Work out the finished part from the listing and answer in its coordinate system (mm). Face numbers are marked on the shaded views. A direction names the side the tool comes from. Coordinates: 2 decimals unless noted, no trailing zeros. Order: outer loops, then holes, each group sorted by start corner. A loop starts at its lowest first (then second) coordinate and runs counter-clockwise, first axis right, second up. Notation, with made-up numbers: (29.25, 6.5) -> (71.25, 6.5) arc R26 ccw to (71.25, 39.5) -> close; hole circle Ø8 at (41.5, 15.5). An arc over 180 degrees is marked (long way). Write item = value, one per line. Start each with the question number.
Q1. Flat-ended cylindrical pins translate along their axes: pin 1 (8 mm diameter, centred on y = 36.5, z = 29.5, fed in from +X); pin 2 (4 mm diameter, centred on x = 18.5, y = 35, fed in from +Z). Find the tip coordinate at first contact, or state that the pin passes through.
Q2. The part is cut by section A-A, the plane y = 29. Determine the outline of the cut face in (x, z), plus the area to 3 significant figures.
Q3. The part is cut by section D-D, the plane y = 50. Determine the outline of the cut face in (x, z), plus the area to 3 significant figures.
Q4. Which of the six approach directions +Z, -Z, +X, -X, +Y, -Y give full straight-line access (tool end or side, diameter ignored) to the marked faces 5 and 6?
Q5. The part is cut by section C-C, the plane z = 7.5. Determine the outline of the cut face in (x, y).
Q6. For a pull along Y with two mould halves and no side action, classify the marked faces 1, 2, 3 and 4 as +Y half, -Y half, draft (parallel to the pull), parting line (faces both ways), or undercut.
Q7. Straight lines are drawn through the part: L1, parallel to Y at x = 39, z = 3; L2, parallel to X at y = 52.5, z = 24.5; L3, parallel to Z at x = 35, y = 3.5. For each, find the intervals that lie inside material, in ascending order. Write a range as from..to.
Q8. The part is cut by section B-B, the plane x = 39. Determine the outline of the cut face in (y, z), plus the area to 3 significant figures.
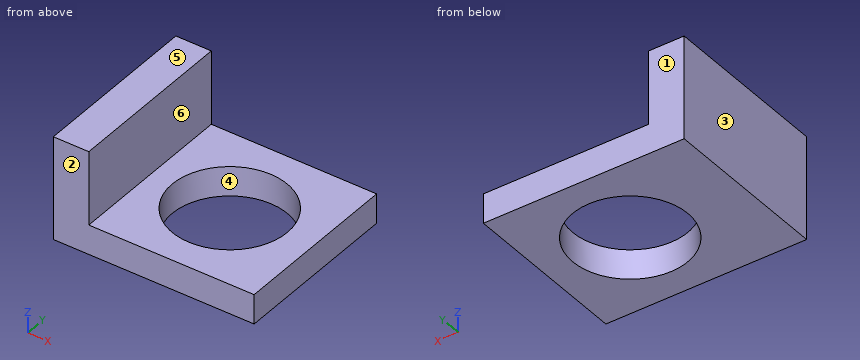
```python
from build123d import *

# Parameters (mm, degrees)
SKETCH_1_W          = 68
SKETCH_1_H          = 58
EXTRUDE_1_DEPTH     = 10
CUT_EXTRUDE_1_REACH = 91.933
SKETCH_2_R          = 19.5
SKETCH_4_W          = 12
SKETCH_4_H          = 58
EXTRUDE_3_DEPTH     = 25


with BuildPart() as part:
    # 草图1 → 凸台-拉伸1 (new body)
    with BuildSketch(Plane.XY):
        with Locations((34, 29)):
            Rectangle(SKETCH_1_W, SKETCH_1_H)
    extrude(amount=EXTRUDE_1_DEPTH)

    # 草图2 → 切除-拉伸1 (cut, up to next)
    with BuildSketch(Plane.XY.offset(10), mode=Mode.PRIVATE) as cut_extrude_1_sk1:
        with Locations((39, 29)):
            Circle(SKETCH_2_R)
    cut_extrude_1_tool1 = extrude(cut_extrude_1_sk1.sketch, amount=-CUT_EXTRUDE_1_REACH, mode=Mode.PRIVATE) & part.part
    add(cut_extrude_1_tool1.solids().sort_by_distance((39, 29, 10))[0], mode=Mode.SUBTRACT)

    # 草图4 → 凸台-拉伸3 (add)
    with BuildSketch(Plane.XY.offset(10)):
        with Locations((6, 29)):
            Rectangle(SKETCH_4_W, SKETCH_4_H)
    extrude(amount=EXTRUDE_3_DEPTH)


solid = part.part
```
Model answer:
q1.pin_1 = 12
q1.pin_2 = 10
q2.outline = (0, 0) -> (19.5, 0) -> (19.5, 10) -> (12, 10) -> (12, 35) -> (0, 35) -> close; (58.5, 0) -> (68, 0) -> (68, 10) -> (58.5, 10) -> close
q2.area = 590 mm2
q3.outline = (0, 0) -> (68, 0) -> (68, 10) -> (12, 10) -> (12, 35) -> (0, 35) -> close
q3.area = 980 mm2
q4.face_5 = +Z, +X, -X, +Y, -Y
q4.face_6 = +Z, +X, +Y, -Y
q5.outline = (0, 0) -> (68, 0) -> (68, 58) -> (0, 58) -> close; hole circle Ø39 at (39, 29)
q6.face_1 = +Y half
q6.face_2 = -Y half
q6.face_3 = draft
q6.face_4 = undercut
q7.L1 = 0..9.5, 48.5..58
q7.L2 = 0..12
q7.L3 = 0..10
q8.outline = (0, 0) -> (9.5, 0) -> (9.5, 10) -> (0, 10) -> close; (48.5, 0) -> (58, 0) -> (58, 10) -> (48.5, 10) -> close
q8.area = 190 mm2
